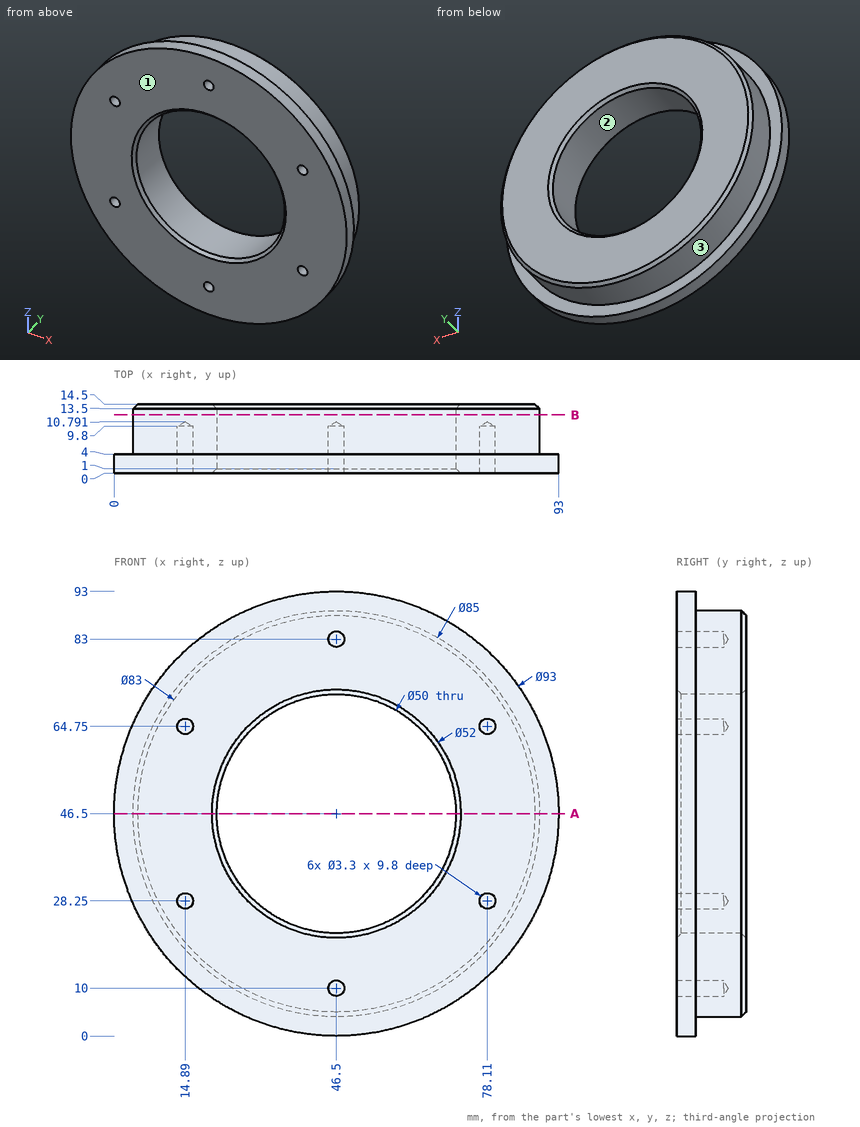
Check sheet for the drawn part. Datum: minimum x, y, z corner. Units: mm. Round coordinates to 2 decimals unless told otherwise and drop trailing zeros. Loops run counter-clockwise (first coordinate to the right, second up) from the corner with the lowest first, then second, coordinate; pieces in that order, holes last. Notation, with made-up numbers: (37.5, 87) - (74.5, 87) arc R11 cw to (74.5, 94) - close; hole circle Ø9 at (-1, 69.5). An arc over 180 degrees is marked (long way). Answer as a JSON object with one key per item and string values. Group by question number.
Q1. Gauge pin test, flat ends, axial feed: P1, Ø4, axis at y = 12, z = 56.5, coming from the -X side; P2, Ø5.5, axis at x = 78.11, z = 28.25, coming from the -Y side; P3, Ø5, axis at x = 61.5, y = 3.5, coming from the +Z side; P4, Ø3, axis at x = 79.5, z = 12, coming from the +Y side. Record the tip position at first contact, or that the pin passes through.
Q2. Mould release check, pull along Z, two halves, no side actions. Record for the marked faces 1, 2 and 3: released by +Z, released by -Z, zero draft, split by the parting line, or undercut.
Q3. Scan lines: line 1 along X through (y, z) = (7.5, 64.75) (1 decimal); line 2 along Z through (x, y) = (77.5, 8) (1 decimal); line 3 along Y through (x, z) = (11, 71). Record each from-to range of solid material in increasing order. Write a range as [from, to].
Q4. Sectioned sample at A-A, the plane z = 46.5. Enter the section's corners in (x, y).
Q5. Sectioned sample at B-B, the plane y = 12.25. Enter the section's corners in (x, z).
Solution:
{
 "1": {"P1": "stops at x = 4.76", "P2": "stops at y = 0", "P3": "stops at z = 91.29", "P4": "stops at y = 4"},
 "2": {"face 1": "zero draft", "face 2": "undercut", "face 3": "split by the parting line"},
 "3": {"line 1": "x = [8.1, 13.2], [16.5, 29.4], [63.6, 76.5], [79.8, 84.9]", "line 2": "z = [17.4, 26.7], [29.8, 63.2], [66.3, 75.6]", "line 3": "y = [0, 4]"},
 "4": {"outline": "(0, 0) - (20.5, 0) - (21.5, 1) - (21.5, 13.5) - (20.5, 14.5) - (5, 14.5) - (4, 13.5) - (4, 4) - (0, 4) - close; (71.5, 1) - (72.5, 0) - (93, 0) - (93, 4) - (89, 4) - (89, 13.5) - (88, 14.5) - (72.5, 14.5) - (71.5, 13.5) - close"},
 "5": {"outline": "circle Ø85 at (46.5, 46.5); hole circle Ø50 at (46.5, 46.5)"}
}
